from build123d import *

# Parameters (mm, degrees)
BOSS_EXTRUDE1_DEPTH = 45
CUT_EXTRUDE1_DEPTH  = 72.788216303
SKETCH3_W           = 11.06
SKETCH3_H           = 58.56
BOSS_EXTRUDE2_DEPTH = 2.5
SKETCH4_W           = 13.06
SKETCH4_H           = 60.56
BOSS_EXTRUDE3_DEPTH = 2.5


with BuildPart() as part:
    # Sketch1 → Boss-Extrude1 (new body)
    with BuildSketch(Plane(origin=(0, 0, 0), x_dir=(1, 0, 0), z_dir=(0, 1, 0))):
        Polygon((-4.14, 27.89), (-4.14, -27.89), (-2.36, -27.89), (-2.36, -23.89), (-1.36, -23.89), (-1.36, -20.89), (1.36, -20.89), (1.36, -23.89), (2.36, -23.89), (2.36, -27.89), (4.14, -27.89), (4.14, 27.89), (2.36, 27.89), (2.36, 23.89), (1.36, 23.89), (1.36, 20.89), (-1.36, 20.89), (-1.36, 23.89), (-2.36, 23.89), (-2.36, 27.89), align=None)
    extrude(amount=BOSS_EXTRUDE1_DEPTH)

    # Sketch2 → Cut-Extrude1 (cut, through all)
    with BuildSketch(Plane.XY.offset(27.89)):
        Polygon((-4.14, 0), (4.14, 0), (4.14, 1.4599874), align=None)
    extrude(amount=-CUT_EXTRUDE1_DEPTH, mode=Mode.SUBTRACT)

    # Sketch3 → Boss-Extrude2 (add)
    with BuildSketch(Plane(origin=(0, 45, 0), x_dir=(1, 0, 0), z_dir=(0, 1, 0))):
        Rectangle(SKETCH3_W, SKETCH3_H)
    extrude(amount=BOSS_EXTRUDE2_DEPTH)

    # Sketch4 → Boss-Extrude3 (add)
    with BuildSketch(Plane(origin=(0, 47.5, 0), x_dir=(1, 0, 0), z_dir=(0, 1, 0))):
        Rectangle(SKETCH4_W, SKETCH4_H)
    extrude(amount=BOSS_EXTRUDE3_DEPTH)


solid = part.part
Build history of the part. All positions in model axes, mm. A direction names the side the tool comes from. Give positions to 0.01 mm unless a question says otherwise; leave off trailing zeros. Write each loop counter-clockwise with the first axis right and the second up, starting at its lowest first coordinate (ties: lowest second). Pieces come first, ordered by that corner, then holes. Notation, with made-up numbers: (-29, 84.5) - (8, 84.5) arc R30 ccw to (8, 115.5) - close; hole circle Ø9 at (-22.5, -8.75). An arc over 180 degrees is marked (long way). Use one line per item in the form item = value. Start each with the question number.
1. Probe line 1 (X direction, y = 35.5, z = -23); line 2 (X direction, y = 37, z = -2.5); line 3 (Z direction, x = 4, y = 32). List the from-to ranges inside material, lowest first. Write a range as [from, to].
2. Band-saw the part on A-A on z = 25.5. Write the cut outline in (x, y).
3. Two-plate mould, pull along X, no slides. Class faces 1 (the face through (3, 23, -27.89)), 2 (the face through (-4.14, 22, 0)), 3 (the face through (1.36, 23, -22)), 4 (the face through (1.36, 23, 22)): released by +X, released by -X, zero draft, split by the parting line, or undercut.
4. Drop flat-ended pins along their axis: pin 1 Ø0.5 at (x, y) = (-2, 32) entering from +Z; pin 2 Ø3.5 at (y, z) = (33.5, 22.5) entering from -X; pin 3 Ø1.4 at (x, y) = (3, 28.5) entering from -Z. Give the stop position or say it passes through.
5. Band-saw the part on D-D on z = -7.5. Write the cut outline in (x, y), plus the area to 3 significant figures.
6. 3-axis set-ups, long thin cutter, end or side, ignore diameter. For faces 5 (the face through (4.14, 23, 0)), 6 (the face through (0, 50, 0)), 7 (the face through (0, 46, 29.28)), 8 (the face through (2.36, 23, 26)), 9 (the face through (-1.36, 22, -22)): which of +Z, -Z, +X, -X, +Y, -Y reach the whole face in a straight line?
7. Band-saw the part on B-B on y = 12.5. Write the cut outline in (x, z), plus the area to 3 significant figures.
8. Band-saw the part on C-C on x = 0. Write the cut outline in (y, z).
Conclusion:
q1.line_1 = [-4.14, -1.36], [1.36, 4.14]
q1.line_2 = [-4.14, 4.14]
q1.line_3 = [-27.89, 27.89]
q2.outline = (-6.53, 47.5) - (-5.53, 47.5) - (-5.53, 45) - (-4.14, 45) - (-4.14, 0) - (-2.36, 0.31) - (-2.36, 45) - (2.36, 45) - (2.36, 1.15) - (4.14, 1.46) - (4.14, 45) - (5.53, 45) - (5.53, 47.5) - (6.53, 47.5) - (6.53, 50) - (-6.53, 50) - close
q3.face_1 = zero draft
q3.face_2 = released by -X
q3.face_3 = undercut
q3.face_4 = undercut
q4.pin_1 = 23.89
q4.pin_2 = -4.14
q4.pin_3 = -27.89
q5.outline = (-6.53, 47.5) - (-5.53, 47.5) - (-5.53, 45) - (-4.14, 45) - (-4.14, 0) - (4.14, 1.46) - (4.14, 45) - (5.53, 45) - (5.53, 47.5) - (6.53, 47.5) - (6.53, 50) - (-6.53, 50) - close
q5.area = 427 mm²
q6.face_5 = +Z, -Z, +X, -Y
q6.face_6 = +Z, -Z, +X, -X, +Y
q6.face_7 = +Z, +X, -X, -Y
q6.face_8 = +Z, -Y
q6.face_9 = -Z, -Y
q7.outline = (-4.14, -27.89) - (-2.36, -27.89) - (-2.36, -23.89) - (-1.36, -23.89) - (-1.36, -20.89) - (1.36, -20.89) - (1.36, -23.89) - (2.36, -23.89) - (2.36, -27.89) - (4.14, -27.89) - (4.14, 27.89) - (2.36, 27.89) - (2.36, 23.89) - (1.36, 23.89) - (1.36, 20.89) - (-1.36, 20.89) - (-1.36, 23.89) - (-2.36, 23.89) - (-2.36, 27.89) - (-4.14, 27.89) - close
q7.area = 408 mm²
q8.outline = (0.73, -20.89) - (45, -20.89) - (45, -29.28) - (47.5, -29.28) - (47.5, -30.28) - (50, -30.28) - (50, 30.28) - (47.5, 30.28) - (47.5, 29.28) - (45, 29.28) - (45, 20.89) - (0.73, 20.89) - close
